Verification items for the finished model (mm, model axes). A direction names the side the tool comes from. Round coordinates to 2 decimals unless told otherwise and drop trailing zeros. Write each loop counter-clockwise with the first axis right and the second up, starting at its lowest first coordinate (ties: lowest second). Pieces come first, ordered by that corner, then holes.
from build123d import *

# Parameters (mm, degrees)
SKETCH_1_R               = 50
SKETCH_1_W               = 5.2
SKETCH_1_H               = 30
EXTRUDE_1_DEPTH          = 5
SKETCH_2_R               = 60
SKETCH_2_W               = 5.2
SKETCH_2_H               = 30
EXTRUDE_2_DEPTH          = 10
CUT_EXTRUDE_START        = -10
SKETCH_4_R               = 60
CUT_EXTRUDE_1_DEPTH      = 10
SKETCH_8_W               = 5.2
SKETCH_8_H               = 30
EXTRUDE_5_DEPTH          = 20
SKETCH_6_R               = 2.2
CUT_EXTRUDE_2_DEPTH      = 42
PATTERN_CIRCULAR_1_COUNT = 3
SKETCH_9_R               = 2.75
CUT_EXTRUDE_3_DEPTH      = 10
SKETCH_10_R              = 6
CUT_EXTRUDE_4_DEPTH      = 0.5
PATTERN_CIRCULAR_2_COUNT = 3


with BuildPart() as part:
    # 草图1 → 凸台-拉伸1 (new body)
    with BuildSketch(Plane.XY):
        Circle(SKETCH_1_R)
        with Locations((0, 22)):
            Rectangle(SKETCH_1_W, SKETCH_1_H, mode=Mode.SUBTRACT)
        Polygon((4.762177826, -5.75166605), (30.74293994, -20.75166605), (33.34293994, -16.24833395), (7.362177826, -1.24833395), align=None, mode=Mode.SUBTRACT)
        Polygon((-7.362177826, -1.24833395), (-33.34293994, -16.24833395), (-30.74293994, -20.75166605), (-4.762177826, -5.75166605), align=None, mode=Mode.SUBTRACT)
    extrude(amount=EXTRUDE_1_DEPTH)

    # 草图2 → 凸台-拉伸2 (add)
    with BuildSketch(Plane.XY):
        Circle(SKETCH_2_R)
        with Locations((0, 22)):
            Rectangle(SKETCH_2_W, SKETCH_2_H, mode=Mode.SUBTRACT)
        Polygon((7.362177826, -1.24833395), (4.762177826, -5.75166605), (30.74293994, -20.75166605), (33.34293994, -16.24833395), align=None, mode=Mode.SUBTRACT)
        Polygon((-4.762177826, -5.75166605), (-7.362177826, -1.24833395), (-33.34293994, -16.24833395), (-30.74293994, -20.75166605), align=None, mode=Mode.SUBTRACT)
    extrude(amount=-EXTRUDE_2_DEPTH)

    # 草图4 → 切除-拉伸1 (cut)
    with BuildSketch(Plane(origin=(0, 0, -10), x_dir=(-1, 0, 0), z_dir=(0, 0, -1)).offset(CUT_EXTRUDE_START)):
        Circle(SKETCH_4_R)
        Polygon((-47.003193978, -12.588079912), (-12.6, 7.274613392), (-12.6, 47), (12.6, 47), (12.6, 7.274613392), (47.003193978, -12.588079912), (34.403193978, -34.411920088), (0, -14.549226784), (-34.403193978, -34.411920088), align=None, mode=Mode.SUBTRACT)
    extrude(amount=CUT_EXTRUDE_1_DEPTH, mode=Mode.SUBTRACT)

    # 草图8 → 凸台-拉伸5 (add)
    with BuildSketch(Plane(origin=(0, 0, -10), x_dir=(-1, 0, 0), z_dir=(0, 0, -1))):
        Polygon((47.003193978, -12.588079912), (12.6, 7.274613392), (12.6, 47), (-12.6, 47), (-12.6, 7.274613392), (-47.003193978, -12.588079912), (-34.403193978, -34.411920088), (0, -14.549226784), (34.403193978, -34.411920088), align=None)
        with Locations((0, 22)):
            Rectangle(SKETCH_8_W, SKETCH_8_H, mode=Mode.SUBTRACT)
        Polygon((-4.762177826, -5.75166605), (-7.362177826, -1.24833395), (-33.34293994, -16.24833395), (-30.74293994, -20.75166605), align=None, mode=Mode.SUBTRACT)
        Polygon((7.362177826, -1.24833395), (4.762177826, -5.75166605), (30.74293994, -20.75166605), (33.34293994, -16.24833395), align=None, mode=Mode.SUBTRACT)
    extrude(amount=EXTRUDE_5_DEPTH)

    # 草图6 → 切除-拉伸2 (cut)
    with BuildSketch(Plane(origin=(6.3, -10.911920088, 0), x_dir=(0.8660254037844384, 0.5000000000000004, 0), z_dir=(0.5000000000000004, -0.8660254037844384, 0))):
        with Locations((-30, -20)):
            Circle(SKETCH_6_R)
        with Locations((-14, -20)):
            Circle(SKETCH_6_R)
    cut_extrude_2 = extrude(amount=-CUT_EXTRUDE_2_DEPTH, mode=Mode.SUBTRACT)

    # 阵列(圆周)1: 切除-拉伸2 ×3 about axis
    pattern_circular_1_axis = Axis((0, 0, 5), (0, 0, -1))
    for i in range(1, PATTERN_CIRCULAR_1_COUNT):
        add(cut_extrude_2.rotate(pattern_circular_1_axis, i * 360 / PATTERN_CIRCULAR_1_COUNT), mode=Mode.SUBTRACT)

    # 草图9 → 切除-拉伸3 (cut)
    with BuildSketch(Plane(origin=(0, 0, 0), x_dir=(-1, 0, 0), z_dir=(0, 0, -1))):
        with Locations((28.284271247, 28.284271247)):
            Circle(SKETCH_9_R)
        with Locations((38.637033052, 10.352761804)):
            Circle(SKETCH_9_R)
    cut_extrude_3 = extrude(amount=-CUT_EXTRUDE_3_DEPTH, mode=Mode.SUBTRACT)

    # 草图10 → 切除-拉伸4 (cut)
    with BuildSketch(Plane(origin=(0, 0, 0), x_dir=(-1, 0, 0), z_dir=(0, 0, -1))):
        with Locations((28.284271247, 28.284271247)):
            Circle(SKETCH_10_R)
        with Locations((38.637033052, 10.352761804)):
            Circle(SKETCH_10_R)
    cut_extrude_4 = extrude(amount=-CUT_EXTRUDE_4_DEPTH, mode=Mode.SUBTRACT)

    # 阵列(圆周)2: 切除-拉伸3, 切除-拉伸4 ×3 about axis
    pattern_circular_2_axis = Axis((0, 0, 0), (0, 0, 1))
    add([cut_extrude_3.rotate(pattern_circular_2_axis, i * 360 / PATTERN_CIRCULAR_2_COUNT) for i in range(1, PATTERN_CIRCULAR_2_COUNT)], mode=Mode.SUBTRACT)
    add([cut_extrude_4.rotate(pattern_circular_2_axis, i * 360 / PATTERN_CIRCULAR_2_COUNT) for i in range(1, PATTERN_CIRCULAR_2_COUNT)], mode=Mode.SUBTRACT)


solid = part.part
Q1. Sectioned sample at A-A (y = 41.5). Enter the section's corners in (x, z).
Recorded:
outline: (-27.89, 0) - (-12.6, 0) - (-12.6, -30) - (12.6, -30) - (12.6, 0) - (27.89, 0) - (27.89, 5) - (-27.89, 5) - close
Q2. Depth check by flat-ended pin: P1, Ø6, axis at x = -13, y = -37, coming from the -Z side; P2, Ø9.5, axis at x = -39, y = 11, coming from the -Z side; P3, Ø7.5, axis at x = 3.5, z = -13, coming from the +Y side; P4, Ø2, axis at y = -37, z = -17.5, coming from the -X side. Enter the tip coordinate at first touch or a pass-through.
Recorded:
P1: stops at z = 0
P2: stops at z = 0.5
P3: stops at y = 47
P4: passes through
Q3. Sectioned sample at B-B (y = 0). Give the number of separate pieces and of enclosed holes in the cut face, plus the area to 3 significant figures.
Recorded:
separate pieces: 1
enclosed holes: 2
area: 1,980 mm2
Q4. Release check for a two-part mould opening along Z. For faces 1 (the flat face through (17.934, -13.357, -12.255)), 2 (the cylindrical face through (16.372, -0.596, -22.148)), 3 (the flat face through (1, -2, -30)), 4 (the cylindrical face through (-7.67, 11.9, -19.34)) record: released by +Z, released by -Z, zero draft, split by the parting line, or undercut.
Recorded:
face 1: zero draft
face 2: undercut
face 3: released by -Z
face 4: undercut
Q5. Material ranges on line 1 along Y through (x, z) = (-11.5, 3); line 2 along Z through (x, y) = (-7.75, 14); line 3 along X through (y, z) = (-10, -2.5), recorded low to high.
Recorded:
line 1: y = -48.66 to -41.14, -36.14 to -9.64, -3.64 to 48.66
line 2: z = -30 to -22.2, -17.8 to 5
line 3: x = -42.52 to -22.52, -12.12 to 12.12, 22.52 to 42.52
Q6. Tool access check on faces 5 (the flat face through (0, 37, -12)), 6 (the flat face through (-40.615, -23.653, -14.79)), 7 (the flat face through (-16.96, -24.34, -14.79)), 8 (the flat face through (1, -22, 0)). Record the directions out of +Z, -Z, +X, -X, +Y, -Y that give a thin tool (end or side, any length) a straight path to the whole face; none if there is none.
Recorded:
face 5: +Z, -Z
face 6: -Z, -X, -Y
face 7: -Z, -Y
face 8: -Z
